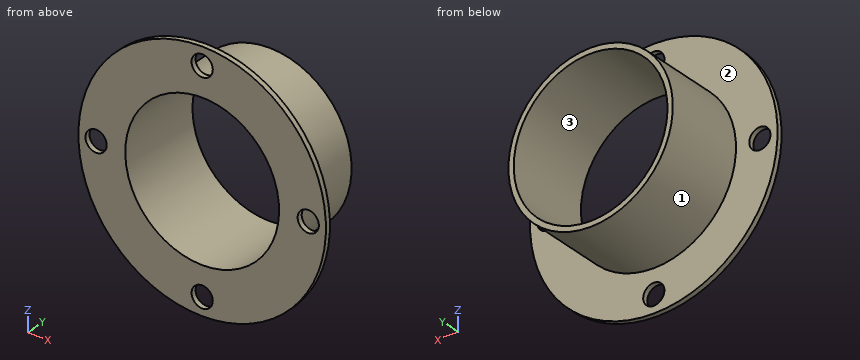
```python
from build123d import *

# Parameters (mm, degrees)
SKETCH_2_R          = 6
CUT_EXTRUDE_1_DEPTH = 110.585582993


with BuildPart() as part:
    # 草图1 → 旋转1 (revolve)
    with BuildSketch(Plane.XY, mode=Mode.PRIVATE) as revolve_1_sk:
        Polygon((43.5, 50), (43.5, 0), (70, 0), (70, 3), (46.5, 3), (46.5, 50), align=None)
    revolve(revolve_1_sk.sketch.rotate(Axis((0, 0, 0), (0, 1, 0)), 90), axis=Axis((0, 0, 0), (0, 1, 0)))

    # 草图2 → 切除-拉伸1 (cut, through all)
    with BuildSketch(Plane(origin=(0, 3, 0), x_dir=(1, 0, 0), z_dir=(0, 1, 0))):
        with Locations(Location((0, 60, 0), (0, 0, 270))):
            Circle(SKETCH_2_R)
        with Locations(Location((60, 0, 0), (0, 0, 270))):
            Circle(SKETCH_2_R)
        with Locations(Location((0, -60, 0), (0, 0, 270))):
            Circle(SKETCH_2_R)
        with Locations(Location((-60, 0, 0), (0, 0, 270))):
            Circle(SKETCH_2_R)
    extrude(amount=-CUT_EXTRUDE_1_DEPTH, mode=Mode.SUBTRACT)


solid = part.part
```
Read the model definition and answer for the solid it produces. Units are mm, in the model's axes. Face numbers are marked on the shaded views. Coordinates: 2 decimals unless noted, no trailing zeros. Loops run counter-clockwise (first coordinate to the right, second up) from the corner with the lowest first, then second, coordinate; pieces in that order, holes last. Notation, with made-up numbers: (-21.75, 25) - (8.25, 25) arc R20 cw to (8.25, 44) - close; hole circle Ø4 at (10, 53.5). An arc over 180 degrees is marked (long way). Answer in a Markdown table with one row per item.
1. Find section C-C, the plane y = 7. Write down the section's boundary in (x, z), then the cut area to 3 significant figures.
Conclusion:
| item | result |
|---|---|
| outline | circle Ø93 at (0, 0); hole circle Ø87 at (0, 0) |
| area | 848 mm² |
2. Find section B-B, the plane z = -35.5. Write down the section's boundary in (x, y), then the cut area to 3 significant figures.
Conclusion:
| item | result |
|---|---|
| outline | (-60.33, 0) - (-25.14, 0) - (-25.14, 50) - (-30.03, 50) - (-30.03, 3) - (-60.33, 3) - close; (25.14, 0) - (60.33, 0) - (60.33, 3) - (30.03, 3) - (30.03, 50) - (25.14, 50) - close |
| area | 671 mm² |
3. Find section D-D, the plane x = -60. Write down the section's boundary in (y, z), then the cut area to 3 significant figures.
Conclusion:
| item | result |
|---|---|
| outline | (0, -36.06) - (3, -36.06) - (3, -6) - (0, -6) - close; (0, 6) - (3, 6) - (3, 36.06) - (0, 36.06) - close |
| area | 180 mm² |
4. Straight lines are drawn through the part: line 1 (Z direction, x = 1, y = 31.5); line 2 (X direction, y = 39.5, z = 0); line 3 (Y direction, x = -28, z = -51.5). For each, find the intervals that lie inside material, in ascending order.
Conclusion:
| item | result |
|---|---|
| line 1 | z = -46.49 to -43.49, 43.49 to 46.49 |
| line 2 | x = -46.5 to -43.5, 43.5 to 46.5 |
| line 3 | y = 0 to 3 |
5. Find section A-A, the plane x = 0. Write down the section's boundary in (y, z).
Conclusion:
| item | result |
|---|---|
| outline | (0, -70) - (3, -70) - (3, -66) - (0, -66) - close; (0, -54) - (3, -54) - (3, -46.5) - (50, -46.5) - (50, -43.5) - (0, -43.5) - close; (0, 43.5) - (50, 43.5) - (50, 46.5) - (3, 46.5) - (3, 54) - (0, 54) - close; (0, 66) - (3, 66) - (3, 70) - (0, 70) - close |
6. Given pin 1 (4 mm diameter, centred on y = 21, z = -21.5, fed in from -X); pin 2 (2 mm diameter, centred on x = 32, y = 37, fed in from +Z); pin 3 (6 mm diameter, centred on y = 19.5, z = 14, fed in from -X), each flat-ended and moving along its own axis, determine where each tip first touches the part or whether it passes through.
Conclusion:
| item | result |
|---|---|
| pin 1 | stops at x = -42.21 |
| pin 2 | stops at z = 34.66 |
| pin 3 | stops at x = -45.18 |
7. Determine the mould class of the marked faces 1, 2 and 3 for opening direction Z: +Z half, -Z half, draft (parallel to the pull), parting line (faces both ways), or undercut.
Conclusion:
| item | result |
|---|---|
| face 1 | parting line |
| face 2 | draft |
| face 3 | undercut |
